Could you check a few things on this drawing? It's one solid part, dimensions in mm from its lowest x, y, z. A direction names the side the tool comes from. Coordinates: 2 decimals unless noted, no trailing zeros. Order: outer loops, then holes, each group sorted by start corner. A loop starts at its lowest first (then second) coordinate and runs counter-clockwise, first axis right, second up.
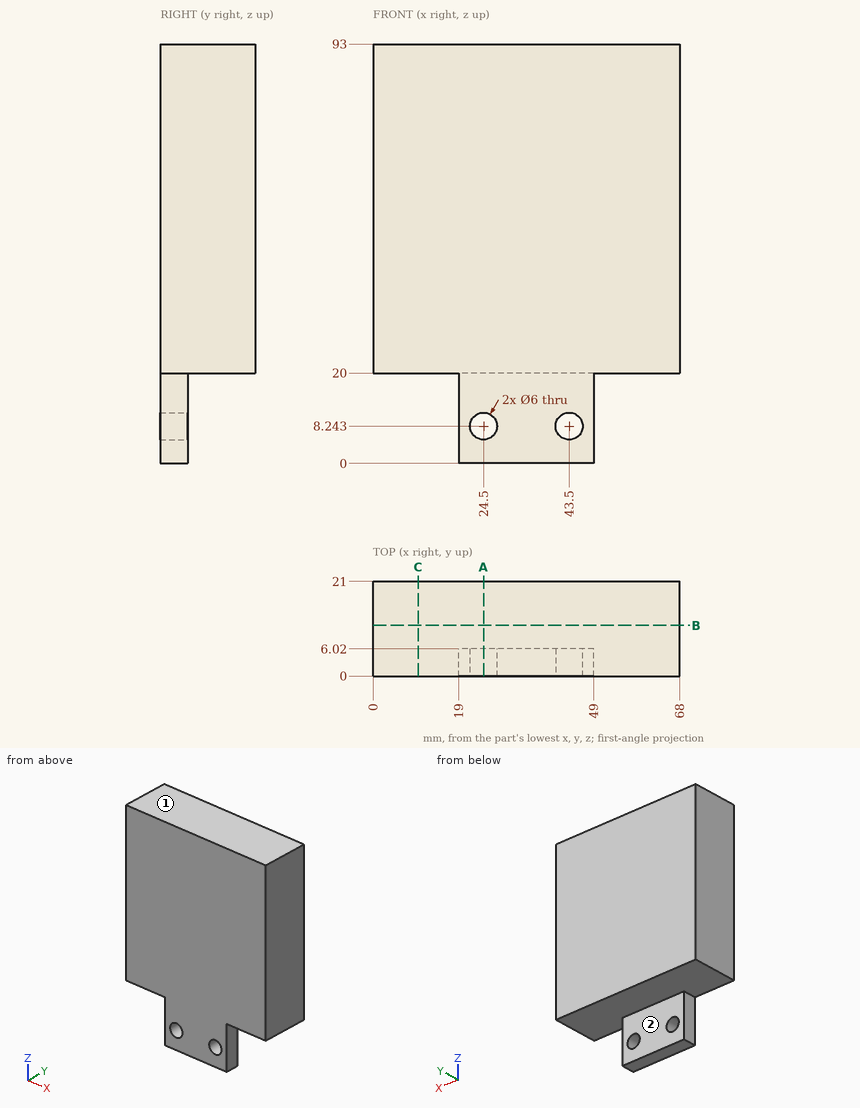
Q1. Will these pins go through, and if not, where does the flat tip stop? pin 1 (3 mm diameter, centred on x = 60, y = 8, fed in from -Z); pin 2 (16 mm diameter, centred on x = 27, z = 7, fed in from +Y); pin 3 (6.5 mm diameter, centred on y = 4, z = 14.5, fed in from +X); pin 4 (5.5 mm diameter, centred on x = 43.5, z = 8.24, fed in from +Y).
Q2. If we section it at C-C on x = 10: Write out the boundary of the cut face in (y, z), then the cut area to 3 significant figures.
Q3. If we section it at B-B on y = 11.25: Write out the boundary of the cut face in (x, z).
Q4. If we section it at A-A on x = 24.5: Write out the boundary of the cut face in (y, z).
Q5. For the marked faces 1 and 2, which set-ups out of +Z, -Z, +X, -X, +Y, -Y let a thin tool reach every point of the face, with its end or its side?
Q6. I need wall thicknesses on L1, parallel to Z at x = 12, y = 12.5; L2, parallel to Z at x = 43.5, y = 2; L3, parallel to X at y = 3.75, z = 16. Which ranges of each line are inside material? Lowest first, please.
Reply:
1. pin 1: stops at z = 20
1. pin 2: stops at y = 6.02
1. pin 3: stops at x = 49
1. pin 4: passes through
2. outline: (0, 20) - (21, 20) - (21, 93) - (0, 93) - close
2. area: 1,530 mm2
3. outline: (0, 20) - (68, 20) - (68, 93) - (0, 93) - close
4. outline: (0, 0) - (6.02, 0) - (6.02, 5.24) - (0, 5.24) - close; (0, 11.24) - (6.02, 11.24) - (6.02, 20) - (21, 20) - (21, 93) - (0, 93) - close
5. face 1: +Z, +X, -X, +Y, -Y
5. face 2: -Z, +X, -X, +Y
6. L1: z = 20 to 93
6. L2: z = 0 to 5.24, 11.24 to 93
6. L3: x = 19 to 49
